```python
from build123d import *

# Parameters (mm, degrees)
SKETCH_1_R           = 4
EXTRUDE_1_DEPTH      = 20
SKETCH_2_R           = 5
EXTRUDE_2_DEPTH      = 3
SKETCH_3_OUTSIDE_W   = 17.4
SKETCH_3_OUTSIDE_H   = 17.4
SKETCH_3_OUTSIDE_W_2 = 14.173876264
SKETCH_3_OUTSIDE_H_2 = 8
CUT_EXTRUDE_1_DEPTH  = 25.062418831
SKETCH_4_R           = 5
EXTRUDE_3_DEPTH      = 20


with BuildPart() as part:
    # 草图1 → 凸台-拉伸1 (new body)
    with BuildSketch(Plane(origin=(0, 0, 0), x_dir=(0, 0, -1), z_dir=(1, 0, 0))):
        Circle(SKETCH_1_R)
    extrude(amount=EXTRUDE_1_DEPTH)

    # 草图2 → 凸台-拉伸2 (add)
    with BuildSketch(Plane.ZY):
        Circle(SKETCH_2_R)
    extrude(amount=EXTRUDE_2_DEPTH)

    # 草图3 outside → 切除-拉伸1 (cut, through all)
    with BuildSketch(Plane.ZY.offset(3)):
        Rectangle(SKETCH_3_OUTSIDE_W, SKETCH_3_OUTSIDE_H)
        Rectangle(SKETCH_3_OUTSIDE_W_2, SKETCH_3_OUTSIDE_H_2, mode=Mode.SUBTRACT)
    extrude(amount=-CUT_EXTRUDE_1_DEPTH, mode=Mode.SUBTRACT)

    # 草图4 → 凸台-拉伸3 (add)
    with BuildSketch(Plane.ZY.offset(3)):
        with Locations(Location((0, 0, 0), (0, 0, 126.869897646))):
            Circle(SKETCH_4_R)
    extrude(amount=EXTRUDE_3_DEPTH)


solid = part.part
```
Read the model definition and answer for the solid it produces. Units are mm, in the model's axes. A direction names the side the tool comes from. Coordinates: 2 decimals unless noted, no trailing zeros. Loops run counter-clockwise (first coordinate to the right, second up) from the corner with the lowest first, then second, coordinate; pieces in that order, holes last.
(1) A tool of negligible diameter and unlimited length cuts with its end or side. For faces 1 (the face through (9.86, -3.905, 0.867)), 2 (the face through (-2, -4, 0)), 3 (the face through (-3, 4.4, -0.1)), from which of +Z, -Z, +X, -X, +Y, -Y can it reach the whole face along a straight path? Write none if from no direction.
Solution:
face 1: +X
face 2: +Z, -Z, +X, -Y
face 3: +Z, -Z, +X, +Y
(2) The part is cut by section B-B (z = 1.75). Determine the outline of the cut face in (x, y), and give its area (3 significant figures).
Solution:
outline: (-23, -4.68) - (-3, -4.68) - (-3, -4) - (0, -4) - (0, -3.6) - (20, -3.6) - (20, 3.6) - (0, 3.6) - (0, 4) - (-3, 4) - (-3, 4.68) - (-23, 4.68) - close
area: 355 mm2
(3) Flat-ended cylindrical pins translate along their axes: pin 1 Ø1.5 at (x, z) = (-2, -0.5) entering from -Y; pin 2 Ø4 at (x, z) = (6, -1) entering from +Y; pin 3 Ø6 at (x, z) = (-0.5, -2.5) entering from +Y. Find the tip coordinate at first contact, or state that the pin passes through.
Solution:
pin 1: stops at y = -4
pin 2: stops at y = 4
pin 3: stops at y = 4.93
(4) Consider line 1 along X through (y, z) = (2.75, 3); line 2 along Z through (x, y) = (10.5, -0.25); line 3 along Y through (x, z) = (-17, -3). Determine where each line is inside the solid, lowest interval first.
Solution:
line 1: x = -23 to 0
line 2: z = -3.99 to 3.99
line 3: y = -4 to 4
(5) The part is cut by section A-A (y = 0). Determine the outline of the cut face in (x, z).
Solution:
outline: (-23, -5) - (0, -5) - (0, -4) - (20, -4) - (20, 4) - (0, 4) - (0, 5) - (-23, 5) - close
(6) The part is cut by section D-D (y = 3.5). Determine the outline of the cut face in (x, z).
Solution:
outline: (-23, -3.57) - (0, -3.57) - (0, -1.94) - (20, -1.94) - (20, 1.94) - (0, 1.94) - (0, 3.57) - (-23, 3.57) - close
(7) The part is cut by section C-C (x = -12.5). Determine the outline of the cut face in (y, z), and give its area (3 significant figures).
Solution:
outline: circle Ø10 at (0, 0)
area: 78.5 mm2
